CAD build for the part. Positions are in the model's coordinates, mm. A direction names the side the tool comes from. Coordinates: 2 decimals unless noted, no trailing zeros. Order: outer loops, then holes, each group sorted by start corner. A loop starts at its lowest first (then second) coordinate and runs counter-clockwise, first axis right, second up. Notation, with made-up numbers: (-31, 88) - (1, 88) arc R26 cw to (1, 127) - close; hole circle Ø5 at (64.25, 75.25). An arc over 180 degrees is marked (long way). Write each question's results on one line, items separated by ' | '. Start each with the question number.
Q1. Band-saw the part on C-C, the plane x = 38. Write the cut outline in (y, z), then the cut area to 3 significant figures.
Q2. Pull direction X, two halves, no side cores. Call faces 3 (the cylindrical face through (11.923, 3.755, 45.72)), 4 (the cylindrical face through (-34.48, -27.47, 7.89)), 5 (the cylindrical face through (-27.47, 34.48, 7.89)), 6 (the flat face through (-1, -22, 16)): released by +X, released by -X, zero draft, split by the parting line, or undercut.
Q3. Band-saw the part on D-D, the plane y = 43.5. Write the cut outline in (x, z), then the cut area to 3 significant figures.
Q4. Band-saw the part on A-A, the plane z = 54. Write the cut outline in (x, y), then the cut area to 3 significant figures.
Q5. Which spindle directions (+Z, -Z, +X, -X, +Y, -Y) get a long thin tool onto all of the face, cutting with end or side? Do faces 1 (the flat face through (-3.4, 12.3, 26)), 2 (the cylindrical face through (33.554, 31.644, 7.888)). Say none if no direction does.
Q6. Pin check, flat tips, straight feed: P1, Ø1.5, axis at y = 9, z = 15.5, coming from the +X side; P2, Ø10, axis at y = 9, z = 45.5, coming from the -X side; P3, Ø2, axis at x = 9.5, z = 47, coming from the +Y side. Stop position of each tip, or through.
Q7. Wall check: probe 1 along Y at (x, z) = (0, 61.75); probe 2 along Z at (x, y) = (-1, 13); probe 3 along Z at (x, y) = (-8, -27). Give the ranges that are in metal, low to high.
Q8. Band-saw the part on B-B, the plane z = 13.5. Write the cut outline in (x, y), then the cut area to 3 significant figures.
```python
from build123d import *

# Parameters (mm, degrees)
SKETCH_1_R                = 50
EXTRUDE_1_DEPTH           = 16
SKETCH_2_R                = 15
EXTRUDE_2_DEPTH           = 10
SKETCH_3_R                = 12.5
EXTRUDE_3_DEPTH           = 40
HOLE_WIZARD_12_5_12_5_1_D = 12.5
PATTERN_CIRCULAR_1_COUNT  = 4
HOLE_WIZARD_M8_1_D        = 6.8
HOLE_WIZARD_M8_1_DEPTH    = 19.75
HOLE_WIZARD_M8_1_TIP      = 2.042926105
FILLET_1_R                = 5


with BuildPart() as part:
    # 草图1 → 凸台-拉伸1 (new body)
    with BuildSketch(Plane.XY):
        Circle(SKETCH_1_R)
    extrude(amount=EXTRUDE_1_DEPTH)

    # 草图2 → 凸台-拉伸2 (add)
    with BuildSketch(Plane.XY.offset(16)):
        Circle(SKETCH_2_R)
    extrude(amount=EXTRUDE_2_DEPTH)

    # 草图3 → 凸台-拉伸3 (add)
    with BuildSketch(Plane.XY.offset(26)):
        Circle(SKETCH_3_R)
    extrude(amount=EXTRUDE_3_DEPTH)

    # Ø12.5 (12.5) 直径孔1 (through all)
    with Locations(Plane.XY.offset(16)):
        with Locations((-28.284271247, 28.284271247)):
            hole_wizard_12_5_12_5_1 = Hole(HOLE_WIZARD_12_5_12_5_1_D / 2)

    # 阵列(圆周)1: Ø12.5 (12.5) 直径孔1 ×4 about axis
    pattern_circular_1_axis = Axis((0, 0, 0), (0, 0, 1))
    for i in range(1, PATTERN_CIRCULAR_1_COUNT):
        add(hole_wizard_12_5_12_5_1.rotate(pattern_circular_1_axis, i * 360 / PATTERN_CIRCULAR_1_COUNT), mode=Mode.SUBTRACT)

    # M8 螺纹孔1
    with Locations(Plane.XY.offset(66)):
        with Locations((0, 0)):
            Hole(HOLE_WIZARD_M8_1_D / 2, depth=HOLE_WIZARD_M8_1_DEPTH)
            with Locations((0, 0, -(HOLE_WIZARD_M8_1_DEPTH + HOLE_WIZARD_M8_1_TIP / 2))):  # 118° drill point
                Cone(0, HOLE_WIZARD_M8_1_D / 2, HOLE_WIZARD_M8_1_TIP, mode=Mode.SUBTRACT)

    # 圆角1
    fillet_1_edges = [part.edges().sort_by_distance(p)[0] for p in [
        (-15, 0, 16),
    ]]
    fillet(fillet_1_edges, radius=FILLET_1_R)


solid = part.part
```
Results below:
1) outline: (-32.5, 0) - (32.5, 0) - (32.5, 16) - (-32.5, 16) - close | area: 1,040 mm²
2) face 3: split by the parting line | face 4: undercut | face 5: undercut | face 6: zero draft
3) outline: (-24.65, 0) - (24.65, 0) - (24.65, 16) - (-24.65, 16) - close | area: 789 mm²
4) outline: circle Ø25 at (0, 0); hole circle Ø6.8 at (0, 0) | area: 455 mm²
5) face 1: +Z | face 2: +Z, -Z
6) P1: stops at x = 49.31 | P2: stops at x = -11.84 | P3: stops at y = 9.17
7) probe 1: y = -12.5 to -3.4, 3.4 to 12.5 | probe 2: z = 0 to 26 | probe 3: z = 0 to 16
8) outline: circle Ø100 at (0, 0); hole circle Ø12.5 at (-28.28, -28.28); hole circle Ø12.5 at (-28.28, 28.28); hole circle Ø12.5 at (28.28, -28.28); hole circle Ø12.5 at (28.28, 28.28) | area: 7,360 mm²
